Input: part model. Units: mm. Frame: model coordinates. Coordinates: 2 decimals unless noted, no trailing zeros. Loops run counter-clockwise (first coordinate to the right, second up) from the corner with the lowest first, then second, coordinate; pieces in that order, holes last. Notation, with made-up numbers: (-9, 58) -> (8, 58) arc R22 ccw to (8, 64) -> close; hole circle Ø10 at (80, -28). An arc over 180 degrees is marked (long way). Put each result on its own line as item: value. Start each with the question number.
1) Cut plane A-A (z = 5.25). Return the cut outline in (x, y) (1 decimal), plus the area to 4 significant figures.
2) Contact query for flat-ended pins moving along their axis: P1, Ø2, axis at y = 9.5, z = 7.5, coming from the +X side; P2, Ø1, axis at x = -7.5, y = -6, coming from the -Z side; P3, Ø2, axis at y = 8.5, z = 12, coming from the -X side; P4, Ø1.5, axis at x = -3, z = 5, coming from the +Y side. Output: stop coordinate, or through.
3) Material intervals for L1, parallel to X at y = -0.25, z = 13.5; L2, parallel to X at y = 3.25, z = 3.5; L3, parallel to Y at x = -4.75, z = 5, sorted ascending.
4) Pull-direction query (Y, two-part tool) for faces 1 (the flat face through (5.92, -10.44, 7.3)), 2 (the conical face through (0.03, 12.443, 14.544)), 3 (the cylindrical face through (-6.91, 0.3, 7.3)); classes: pulls with the +Y half, pulls with the -Y half, needs draft (parallel to the pull), parting line crosses it, or undercut.
from build123d import *

# Parameters (mm, degrees)
SKETCH_1_R          = 6.9175
EXTRUDE_597_DEPTH   = 14.8
SKETCH_2_OUTSIDE_W  = 118.982
SKETCH_2_OUTSIDE_H  = 122.694
SKETCH_2_OUTSIDE_R  = 12
CUT_EXTRUDE_1_DEPTH = 24.559286916
CUT_EXTRUDE_1_DRAFT = -60
SKETCH_3_OUTSIDE_W  = 118.982
SKETCH_3_OUTSIDE_H  = 122.694
SKETCH_3_OUTSIDE_R  = 12
CUT_EXTRUDE_2_DEPTH = 24.559286916
CUT_EXTRUDE_2_DRAFT = -60


with BuildPart() as part:
    # 草图1 → Extrude 597 (new body)
    with BuildSketch(Plane.XY):
        Polygon((0, 13.856406461), (-12, 6.92820323), (-12, -6.92820323), (0, -13.856406461), (12, -6.92820323), (12, 6.92820323), align=None)
        Circle(SKETCH_1_R, mode=Mode.SUBTRACT)
    extrude(amount=EXTRUDE_597_DEPTH)


with BuildPart() as cut_extrude_1_tool:
    # 草图2 outside → 切除-拉伸1 (with draft: the straight prism first)
    with BuildSketch(Plane(origin=(0, 0, 0), x_dir=(-1, 0, 0), z_dir=(0, 0, -1))):
        Rectangle(SKETCH_2_OUTSIDE_W, SKETCH_2_OUTSIDE_H)
        Circle(SKETCH_2_OUTSIDE_R, mode=Mode.SUBTRACT)
    extrude(amount=-CUT_EXTRUDE_1_DEPTH)
    # 切除-拉伸1: the draft: its side faces are tilted about the plane it starts from
    cut_extrude_1_sides = [cut_extrude_1_tool.faces().sort_by_distance(p)[0] for p in [
        (0, -61.347, 12.279643458),
        (-59.491, 0, 12.279643458),
        (0, 61.347, 12.279643458),
        (59.491, 0, 12.279643458),
        (12, 0, 12.279643458),
    ]]
    draft(cut_extrude_1_sides, Plane(origin=(0, 0, 0), x_dir=(-1, 0, 0), z_dir=(0, 0, -1)), CUT_EXTRUDE_1_DRAFT)


with BuildPart() as part_1:
    add(part.part)

    # 切除-拉伸1: cut by cut_extrude_1_tool
    add(cut_extrude_1_tool.part, mode=Mode.SUBTRACT)


with BuildPart() as cut_extrude_2_tool:
    # 草图3 outside → 切除-拉伸2 (with draft: the straight prism first)
    with BuildSketch(Plane.XY.offset(14.8)):
        Rectangle(SKETCH_3_OUTSIDE_W, SKETCH_3_OUTSIDE_H)
        Circle(SKETCH_3_OUTSIDE_R, mode=Mode.SUBTRACT)
    extrude(amount=-CUT_EXTRUDE_2_DEPTH)
    # 切除-拉伸2: the draft: its side faces are tilted about the plane it starts from
    cut_extrude_2_sides = [cut_extrude_2_tool.faces().sort_by_distance(p)[0] for p in [
        (0, -61.347, 2.520356542),
        (59.491, 0, 2.520356542),
        (0, 61.347, 2.520356542),
        (-59.491, 0, 2.520356542),
        (-12, 0, 2.520356542),
    ]]
    draft(cut_extrude_2_sides, Plane.XY.offset(14.8), CUT_EXTRUDE_2_DRAFT)


with BuildPart() as part_2:
    add(part_1.part)

    # 切除-拉伸2: cut by cut_extrude_2_tool
    add(cut_extrude_2_tool.part, mode=Mode.SUBTRACT)


solid = part_2.part
Results found:
1. outline: (-12, -6.9) -> (0, -13.9) -> (12, -6.9) -> (12, 6.9) -> (0, 13.9) -> (-12, 6.9) -> close; hole circle Ø13.8 at (0, 0)
1. area: 348.5 mm2
2. P1: stops at x = 9.28
2. P2: stops at z = 0
2. P3: stops at x = -11.01
2. P4: stops at y = 12.56
3. L1: x = -12 to -6.91, 6.91 to 12
3. L2: x = -12 to -6.11, 6.11 to 12
3. L3: y = -11.11 to -5.03, 5.03 to 11.11
4. face 1: pulls with the -Y half
4. face 2: pulls with the +Y half
4. face 3: undercut
